```python
from build123d import *

# Parameters (mm, degrees)
SKETCH12_R          = 2.5
MEMBER_1_DEPTH      = 600
CUT_EXTRUDE_1_DEPTH = 301.749064836
SKETCH_7_R          = 5
CUT_EXTRUDE_2_DEPTH = 4.999


with BuildPart() as part:
    # Sketch12 → Member 1 (new body)
    with BuildSketch(Plane(origin=(-300, 0, 0), x_dir=(0, 0, -1), z_dir=(1, 0, 0))):
        with BuildLine():
            Line((-6, -15), (-3.25, -15))
            Line((-3.25, -15), (-3.25, -12.7))
            Line((-3.25, -12.7), (-5.7, -12.7))
            Line((-5.7, -12.7), (-5.7, -7))
            ThreePointArc((-5.7, -7), (0, -4.5), (5.7, -7))
            Line((5.7, -7), (5.7, -12.7))
            Line((5.7, -12.7), (3.25, -12.7))
            Line((3.25, -12.7), (3.25, -15))
            Line((3.25, -15), (6, -15))
            ThreePointArc((6, -15), (7.060660172, -14.560660172), (7.5, -13.5))
            Line((7.5, -13.5), (7.5, 13.5))
            ThreePointArc((7.5, 13.5), (7.060660172, 14.560660172), (6, 15))
            Line((6, 15), (3.25, 15))
            Line((3.25, 15), (3.25, 12.7))
            Line((3.25, 12.7), (5.7, 12.7))
            Line((5.7, 12.7), (5.7, 7))
            ThreePointArc((5.7, 7), (0, 4.5), (-5.7, 7))
            Line((-5.7, 7), (-5.7, 12.7))
            Line((-5.7, 12.7), (-3.25, 12.7))
            Line((-3.25, 12.7), (-3.25, 15))
            Line((-3.25, 15), (-6, 15))
            ThreePointArc((-6, 15), (-7.060660172, 14.560660172), (-7.5, 13.5))
            Line((-7.5, 13.5), (-7.5, -13.5))
            ThreePointArc((-7.5, -13.5), (-7.060660172, -14.560660172), (-6, -15))
        make_face()
        Circle(SKETCH12_R, mode=Mode.SUBTRACT)
    extrude(amount=MEMBER_1_DEPTH)

    # 草图4 → 切除-拉伸1 (cut, through all)
    with BuildSketch(Plane.XY.offset(7.5)):
        Polygon((-300, 15), (-270, -15), (-300, -15), align=None)
        Polygon((300, -15), (300, 15), (270, -15), align=None)
    extrude(amount=-CUT_EXTRUDE_1_DEPTH, mode=Mode.SUBTRACT)

    # 草图7 → 切除-拉伸2 (cut)
    with BuildSketch(Plane.XY.offset(-7.5)):
        with Locations(Location((245, 3, 0), (0, 0, 157.483422962))):
            Circle(SKETCH_7_R)
    extrude(amount=CUT_EXTRUDE_2_DEPTH, mode=Mode.SUBTRACT)


solid = part.part
```
Design review of the part built by this model. Coordinates are the model's own, in mm. A direction names the side the tool comes from. Coordinates: 2 decimals unless noted, no trailing zeros. Order: outer loops, then holes, each group sorted by start corner. A loop starts at its lowest first (then second) coordinate and runs counter-clockwise, first axis right, second up. Notation, with made-up numbers: (83.5, 71.5) - (100.5, 71.5) arc R20 ccw to (100.5, 91.5) - close; hole circle Ø5 at (22, -8.75). An arc over 180 degrees is marked (long way). One line per question, with ' | ' between items.
Q1. Consider section B-B, the plane z = 0. Give the boundary of the cut face in (x, y), then the cut area to 3 significant figures.
Answer key:
outline: (-289.5, 4.5) - (-287.5, 2.5) - (287.5, 2.5) - (289.5, 4.5) - close; (-282.5, -2.5) - (-280.5, -4.5) - (280.5, -4.5) - (282.5, -2.5) - close | area: 2,280 mm2
Q2. Consider section A-A, the plane x = 92. Give the boundary of the cut face in (y, z).
Answer key:
outline: (-15, -6) arc R1.5 ccw to (-13.5, -7.5) - (13.5, -7.5) arc R1.5 ccw to (15, -6) - (15, -3.25) - (12.7, -3.25) - (12.7, -5.7) - (7, -5.7) arc R7.75 cw to (7, 5.7) - (12.7, 5.7) - (12.7, 3.25) - (15, 3.25) - (15, 6) arc R1.5 ccw to (13.5, 7.5) - (-13.5, 7.5) arc R1.5 ccw to (-15, 6) - (-15, 3.25) - (-12.7, 3.25) - (-12.7, 5.7) - (-7, 5.7) arc R7.75 cw to (-7, -5.7) - (-12.7, -5.7) - (-12.7, -3.25) - (-15, -3.25) - close; hole circle Ø5 at (0, 0)
Q3. Clearance check with flat-ended pins moving along their axes: pin 1 Ø6 at (x, z) = (73, -1) entering from +Y; pin 2 Ø3 at (x, z) = (193.5, 1.5) entering from +Y; pin 3 Ø6 at (y, z) = (-11, 4.5) entering from +X; pin 4 Ø0.7 at (x, y) = (-33, -14) entering from +Z. State where each tip first meets the part, or that it passes through.
Answer key:
pin 1: stops at y = 15 | pin 2: stops at y = 5.1 | pin 3: stops at x = 276.75 | pin 4: stops at z = 7.49
Q4. For faces 1 (the flat face through (-4, 0, 7.5)), 2 (the cylindrical face through (-3.9, -4.5, 0.1)), list the 3-axis set-ups (+Z, -Z, +X, -X, +Y, -Y) from which the entire face can be reached by the end or side of a thin tool; tool diameter is ignored.
Answer key:
face 1: +Z, +X, -X, +Y, -Y | face 2: +X, -X
Q5. To check wall thickness, follow line 1 along Z through (x, y) = (49, -8); line 2 along Y through (x, z) = (-59, 0); line 3 along Y through (x, z) = (-30.5, 5.5). State the ranges of each line that lie inside material, in increasing order.
Answer key:
line 1: z = -7.5 to -5.7, 5.7 to 7.5 | line 2: y = -4.5 to -2.5, 2.5 to 4.5 | line 3: y = -15 to -12.7, -6.79 to 6.79, 12.7 to 15
Q6. The part is to be moulded in two halves that separate along X. For faces 3 (the cylindrical face through (243.7, -1.83, -5.04)), 4 (the flat face through (-285, 0, 3)), 5 (the flat face through (285, 0, 3)), 6 (the cylindrical face through (-4.1, 4.5, -0.1)), say which applies: +X half, -X half, draft (parallel to the pull), parting line (faces both ways), or undercut.
Answer key:
face 3: undercut | face 4: -X half | face 5: +X half | face 6: draft
